Check sheet for the modelled part. Datum: model origin and axes. Units: mm. A direction names the side the tool comes from. Give positions to 0.01 mm unless a question says otherwise; leave off trailing zeros. Order: outer loops, then holes, each group sorted by start corner. A loop starts at its lowest first (then second) coordinate and runs counter-clockwise, first axis right, second up.
from build123d import *

# Parameters (mm, degrees)
SKETCH1_W             = 39.8
SKETCH1_H             = 20
BOSS_EXTRUDE1_DEPTH   = 51
SKETCH2_R             = 3
BOSS_EXTRUDE2_DEPTH   = 25.5
M3_TAPPED_HOLE1_D     = 2.5
M3_TAPPED_HOLE1_DEPTH = 7.5
M3_TAPPED_HOLE1_TIP   = 0.751075774
FILLET1_R             = 3


with BuildPart() as part:
    # Sketch1 → Boss-Extrude1 (new body)
    with BuildSketch(Plane.XY):
        Rectangle(SKETCH1_W, SKETCH1_H)
    extrude(amount=BOSS_EXTRUDE1_DEPTH)

    # Sketch2 → Boss-Extrude2 (add, symmetric)
    with BuildSketch(Plane(origin=(0, 0, 0), x_dir=(0, 0, -1), z_dir=(1, 0, 0))):
        with Locations(Location((-43.173636791, 0, 0), (0, 0, 90))):
            Circle(SKETCH2_R)
    extrude(amount=BOSS_EXTRUDE2_DEPTH, both=True)

    # M3 Tapped Hole1
    with Locations(Plane(origin=(12.5, 0, 0), x_dir=(-1, 0, 0), z_dir=(0, 0, -1))):
        with Locations((0, 0), (25, 0), (12.62087232, 0)):
            Hole(M3_TAPPED_HOLE1_D / 2, depth=M3_TAPPED_HOLE1_DEPTH)
            with Locations((0, 0, -(M3_TAPPED_HOLE1_DEPTH + M3_TAPPED_HOLE1_TIP / 2))):  # 118° drill point
                Cone(0, M3_TAPPED_HOLE1_D / 2, M3_TAPPED_HOLE1_TIP, mode=Mode.SUBTRACT)

    # Fillet1
    fillet1_edges = [part.edges().sort_by_distance(p)[0] for p in [
        (0, -10, 51),
        (0, 10, 51),
    ]]
    fillet(fillet1_edges, radius=FILLET1_R)


solid = part.part
1) Set-up check for faces 4 (the face through (-1.37, 0.05, 3.8)), 5 (the face through (-22.661, 1.613, 45.703)), 6 (the face through (22.739, 1.613, 45.703)), 7 (the face through (0, 0, 51)): record each of +Z, -Z, +X, -X, +Y, -Y from which the full face is reachable in a straight line by a thin tool's end or side.
Recorded:
face 4: -Z
face 5: -X
face 6: +X
face 7: +Z, +X, -X, +Y, -Y
2) Section check A-A, the plane z = 3.5. Record the cut outline in (x, y), then the cut area to 3 significant figures.
Recorded:
outline: (-19.9, -10) - (19.9, -10) - (19.9, 10) - (-19.9, 10) - close; hole circle Ø2.5 at (-12.5, 0); hole circle Ø2.5 at (-0.12, 0); hole circle Ø2.5 at (12.5, 0)
area: 781 mm2
3) Section check C-C, the plane z = 41. Record the cut outline in (x, y).
Recorded:
outline: (-25.5, -2.07) - (-19.9, -2.07) - (-19.9, -10) - (19.9, -10) - (19.9, -2.07) - (25.5, -2.07) - (25.5, 2.07) - (19.9, 2.07) - (19.9, 10) - (-19.9, 10) - (-19.9, 2.07) - (-25.5, 2.07) - close
4) Depth check by flat-ended pin: pin 1 Ø1.5 at (x, y) = (-0.12, 0) entering from -Z; pin 2 Ø6 at (y, z) = (-2.5, 17) entering from -X; pin 3 Ø12 at (y, z) = (-8, 16) entering from +X. Enter the tip coordinate at first touch or a pass-through.
Recorded:
pin 1: stops at z = 7.8
pin 2: stops at x = -19.9
pin 3: stops at x = 19.9
5) Material ranges on L1, parallel to X at y = 0, z = 3.75; L2, parallel to X at y = 0.25, z = 5; L3, parallel to Y at x = -12.5, z = 3.75, recorded low to high.
Recorded:
L1: x = -19.9 to -13.75, -11.25 to -1.37, 1.13 to 11.25, 13.75 to 19.9
L2: x = -19.9 to -13.72, -11.28 to -1.35, 1.1 to 11.28, 13.72 to 19.9
L3: y = -10 to -1.25, 1.25 to 10
6) Section check D-D, the plane y = -3.75. Record the cut outline in (x, z), then the cut area to 3 significant figures.
Recorded:
outline: (-19.9, 0) - (19.9, 0) - (19.9, 51) - (-19.9, 51) - close
area: 2,030 mm2
7) Draft check along Y on faces 1 (the face through (0.28, 9.1, 50.14)), 2 (the face through (25.5, 0, 43)), 3 (the face through (-0.07, -0.21, 8.12)). Enter one of: +Y half, -Y half, draft (parallel to the pull), parting line (faces both ways), or undercut.
Recorded:
face 1: +Y half
face 2: draft
face 3: undercut
8) Section check B-B, the plane y = 2. Record the cut outline in (x, z).
Recorded:
outline: (-25.5, 40.94) - (-19.9, 40.94) - (-19.9, 0) - (19.9, 0) - (19.9, 40.94) - (25.5, 40.94) - (25.5, 45.41) - (19.9, 45.41) - (19.9, 51) - (-19.9, 51) - (-19.9, 45.41) - (-25.5, 45.41) - close
